Here's the drawing with two shaded views (mm, measured from the low corner). I have some questions. A direction names the side the tool comes from. Round coordinates to 2 decimals unless told otherwise and drop trailing zeros. Order: outer loops, then holes, each group sorted by start corner. A loop starts at its lowest first (then second) coordinate and runs counter-clockwise, first axis right, second up. Notation, with made-up numbers: (-16.75, 37.25) -> (0.25, 37.25) arc R18 cw to (0.25, 62.25) -> close; hole circle Ø2 at (86.5, -6). An arc over 180 degrees is marked (long way). Answer in a Markdown table with one row per item.
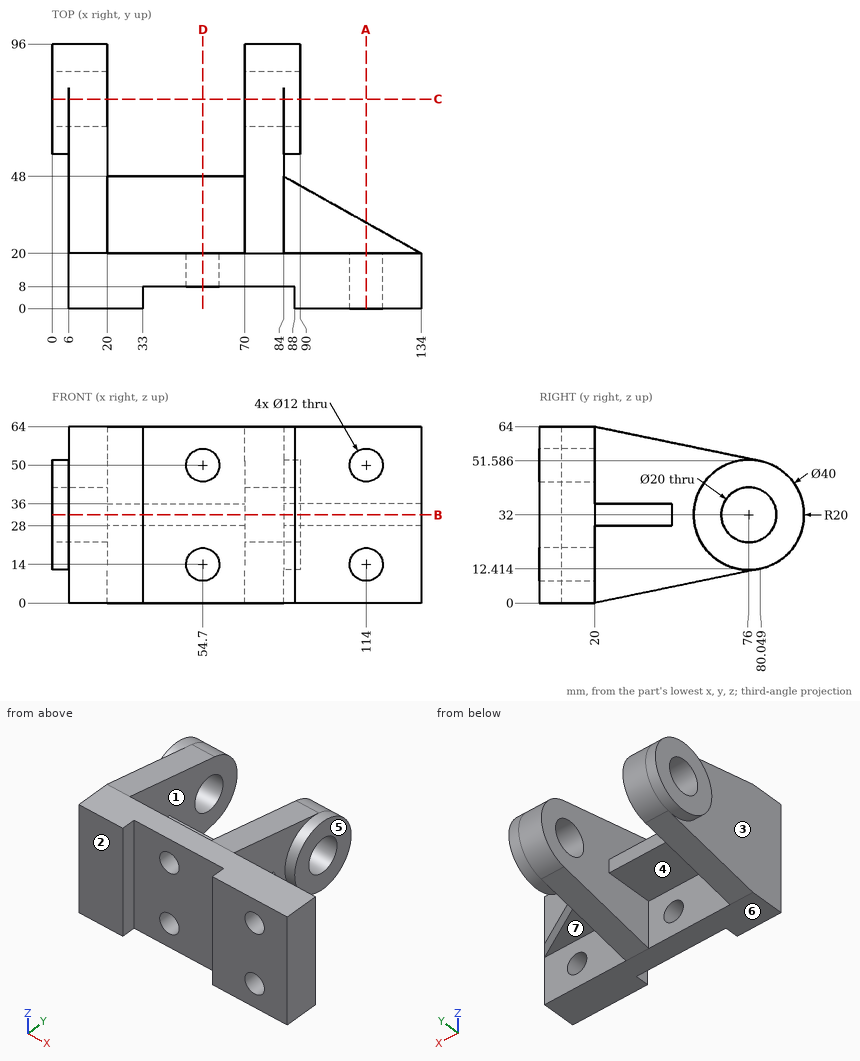
1. Suppose I cut it at C-C on y = 76. Write out the boundary of the cut face in (x, z).
Numbers:
| item | result |
|---|---|
| outline | (0, 12) -> (6, 12) -> (6, 11.58) -> (20, 11.58) -> (20, 22) -> (0, 22) -> close; (0, 42) -> (20, 42) -> (20, 52.42) -> (6, 52.42) -> (6, 52) -> (0, 52) -> close; (70, 11.58) -> (84, 11.58) -> (84, 12) -> (90, 12) -> (90, 22) -> (70, 22) -> close; (70, 42) -> (90, 42) -> (90, 52) -> (84, 52) -> (84, 52.42) -> (70, 52.42) -> close |
2. Please list where these lines run through material, in increasing order: line 1 along X through (y, z) = (9, 14); line 2 along X through (y, z) = (5, 50); line 3 along X through (y, z) = (21.5, 57).
Numbers:
| item | result |
|---|---|
| line 1 | x = 6 to 48.7, 60.7 to 108, 120 to 134 |
| line 2 | x = 6 to 33, 88 to 108, 120 to 134 |
| line 3 | x = 6 to 20, 70 to 84 |
3. We'd pull the mould along X, two halves only. Please class the marked faces 1, 2, 3 and 4: released by +X, released by -X, zero draft, split by the parting line, or undercut.
Numbers:
| item | result |
|---|---|
| face 1 | undercut |
| face 2 | zero draft |
| face 3 | released by -X |
| face 4 | undercut |
4. Suppose I cut it at D-D on x = 54.7. Write out the boundary of the cut face in (y, z).
Numbers:
| item | result |
|---|---|
| outline | (8, 0) -> (20, 0) -> (20, 8) -> (8, 8) -> close; (8, 20) -> (20, 20) -> (20, 28) -> (48, 28) -> (48, 36) -> (20, 36) -> (20, 44) -> (8, 44) -> close; (8, 56) -> (20, 56) -> (20, 64) -> (8, 64) -> close |
5. Suppose I cut it at B-B on z = 32. Write out the boundary of the cut face in (x, y), then the cut area to 3 significant figures.
Numbers:
| item | result |
|---|---|
| outline | (0, 56) -> (6, 56) -> (6, 0) -> (33, 0) -> (33, 8) -> (88, 8) -> (88, 0) -> (134, 0) -> (134, 20) -> (84, 48) -> (84, 56) -> (90, 56) -> (90, 66) -> (70, 66) -> (70, 48) -> (20, 48) -> (20, 66) -> (0, 66) -> close; (0, 86) -> (20, 86) -> (20, 96) -> (0, 96) -> close; (70, 86) -> (90, 86) -> (90, 96) -> (70, 96) -> close |
| area | 6,030 mm2 |
6. For pin 1 Ø8 at (y, z) = (39.5, 44.5) entering from +X; pin 2 Ø20 at (y, z) = (73, 35) entering from +X; pin 3 Ø2.5 at (y, z) = (5.5, 26) entering from -X, each with a flat end and sliding along its axis, tell me the tip position at first contact or that it passes through.
Numbers:
| item | result |
|---|---|
| pin 1 | stops at x = 84 |
| pin 2 | stops at x = 90 |
| pin 3 | stops at x = 6 |
7. Suppose I cut it at A-A on x = 114. Write out the boundary of the cut face in (y, z), then the cut area to 3 significant figures.
Numbers:
| item | result |
|---|---|
| outline | (0, 0) -> (20, 0) -> (20, 8) -> (0, 8) -> close; (0, 20) -> (20, 20) -> (20, 28) -> (31.2, 28) -> (31.2, 36) -> (20, 36) -> (20, 44) -> (0, 44) -> close; (0, 56) -> (20, 56) -> (20, 64) -> (0, 64) -> close |
| area | 890 mm2 |
8. For the marked faces 5, 6 and 7, which set-ups out of +Z, -Z, +X, -X, +Y, -Y let a thin tool reach every point of the face, with its end or its side?
Numbers:
| item | result |
|---|---|
| face 5 | +Z, -Z, +X, +Y |
| face 6 | -Z, +X, -X, +Y, -Y |
| face 7 | -Z, +X |
